The listing builds one solid part. Answer for the finished solid, in the listing's coordinates (mm). A direction names the side the tool comes from. Give positions to 0.01 mm unless a question says otherwise; leave off trailing zeros. Loops run counter-clockwise (first coordinate to the right, second up) from the corner with the lowest first, then second, coordinate; pieces in that order, holes last. Notation, with made-up numbers: M -18.5,31.25 L 32.5,31.25 A20 ccw 32.5,45.25 Z; hole C -6.75,76.25 d4. An arc over 180 degrees is marked long. One line per item, written item: value. Start each with the question number.
Q1. A cutting plane is placed at D-D, the plane z = -24. Determine the outline of the cut face in (x, y).
Q2. A cutting plane is placed at C-C, the plane x = 82. Determine the outline of the cut face in (y, z).
Q3. A cutting plane is placed at B-B, the plane y = 4. State how many separate pieces and enclosed holes the cut face has, and give its area (3 significant figures).
Q4. Consider L1, parallel to X at y = -20, z = 0; L2, parallel to Z at x = -11, y = 2.5; L3, parallel to X at y = -26, z = 4. Determine where each line is inside the solid, lowest interval first.
Q5. The mould has two halves that part along X. Classify faces 4 (the flat face through (90, -12, 0)), 5 (the flat face through (24, -4, -20)), 6 (the cylindrical face through (67.436, -17.675, 0.976)): +X half, -X half, draft (parallel to the pull), parting line (faces both ways), or undercut.
Q6. For faces 1 (the flat face through (26, -20, -24)), 2 (the flat face through (32, 2, 0)), 3 (the cylindrical face through (-17.32, -17.68, 1.63)), determine the directions among +Z, -Z, +X, -X, +Y, -Y from which every point of the face is accessible in a straight line to the end or side of a thin tool.
Q7. A cutting plane is placed at A-A, the plane y = -22. Determine the outline of the cut face in (x, z), and give its area (3 significant figures).
Q8. Flat-ended cylindrical pins translate along their axes: pin 1 (19.5 mm diameter, centred on x = 60, z = 0, fed in from +Y); pin 2 (1 mm diameter, centred on x = 24, y = -23, fed in from -Z); pin 3 (2 mm diameter, centred on x = 39, z = -23.5, fed in from +Y); pin 4 (3 mm diameter, centred on x = 54, y = -22.5, fed in from +Z). Find the tip coordinate at first contact, or state that the pin passes through.
from build123d import *

# Parameters (mm, degrees)
SKETCH1_W           = 180
SKETCH1_H           = 40
BOSS_EXTRUDE1_DEPTH = 6
CUT_EXTRUDE2_DEPTH  = 4
SKETCH6_W           = 180
SKETCH6_H           = 40
BOSS_EXTRUDE3_DEPTH = 30
SKETCH7_W           = 50
SKETCH7_H           = 40
CUT_EXTRUDE3_DEPTH  = 40
SKETCH8_W           = 55
SKETCH8_H           = 10
BOSS_EXTRUDE4_DEPTH = 130
SKETCH9_R           = 7.5
CUT_EXTRUDE4_DEPTH  = 25


with BuildPart() as part:
    # Sketch1 → Boss-Extrude1 (new body)
    with BuildSketch(Plane(origin=(0, 0, 0), x_dir=(1, 0, 0), z_dir=(0, 1, 0))):
        Rectangle(SKETCH1_W, SKETCH1_H)
    extrude(amount=BOSS_EXTRUDE1_DEPTH)

    # Sketch5 → Cut-Extrude2 (cut)
    with BuildSketch(Plane(origin=(0, 6, 0), x_dir=(1, 0, 0), z_dir=(0, 1, 0))):
        with BuildLine():
            Line((-105.561478508, 98.797927369), (119.027484656, -125.791035795))
            ThreePointArc((119.027484656, -125.791035795), (119.027484656, -129.326569701), (115.49195075, -129.326569701))
            Line((115.49195075, -129.326569701), (-109.097012414, 95.262393463))
            ThreePointArc((-109.097012414, 95.262393463), (-109.097012414, 98.797927369), (-105.561478508, 98.797927369))
        make_face()
        with BuildLine():
            Line((-102.025944602, 102.333461275), (122.563018562, -122.255501889))
            ThreePointArc((122.563018562, -122.255501889), (126.098552468, -122.255501889), (126.098552468, -118.719967983))
            Line((126.098552468, -118.719967983), (-98.490410696, 105.868995181))
            ThreePointArc((-98.490410696, 105.868995181), (-102.025944602, 105.868995181), (-102.025944602, 102.333461275))
        make_face()
        with BuildLine():
            Line((-94.95487679, 109.404529087), (129.634086374, -115.184434077))
            ThreePointArc((129.634086374, -115.184434077), (133.16962028, -115.184434077), (133.16962028, -111.648900171))
            Line((133.16962028, -111.648900171), (-91.419342885, 112.940062993))
            ThreePointArc((-91.419342885, 112.940062993), (-94.95487679, 112.940062993), (-94.95487679, 109.404529087))
        make_face()
        with BuildLine():
            Line((-87.883808979, 116.475596899), (136.705154185, -108.113366265))
            ThreePointArc((136.705154185, -108.113366265), (140.240688091, -108.113366265), (140.240688091, -104.577832359))
            Line((140.240688091, -104.577832359), (-84.348275073, 120.011130805))
            ThreePointArc((-84.348275073, 120.011130805), (-87.883808979, 120.011130805), (-87.883808979, 116.475596899))
        make_face()
        with BuildLine():
            Line((-80.812741167, 123.546664711), (143.776221997, -101.042298453))
            ThreePointArc((143.776221997, -101.042298453), (147.311755903, -101.042298453), (147.311755903, -97.506764547))
            Line((147.311755903, -97.506764547), (-77.277207261, 127.082198617))
            ThreePointArc((-77.277207261, 127.082198617), (-80.812741167, 127.082198617), (-80.812741167, 123.546664711))
        make_face()
        with BuildLine():
            Line((-73.741673355, 130.617732523), (150.847289809, -93.971230641))
            ThreePointArc((150.847289809, -93.971230641), (154.382823715, -93.971230641), (154.382823715, -90.435696735))
            Line((154.382823715, -90.435696735), (-70.206139449, 134.153266429))
            ThreePointArc((-70.206139449, 134.153266429), (-73.741673355, 134.153266429), (-73.741673355, 130.617732523))
        make_face()
        with BuildLine():
            Line((-66.670605543, 137.688800335), (157.918357621, -86.900162829))
            ThreePointArc((157.918357621, -86.900162829), (161.453891527, -86.900162829), (161.453891527, -83.364628923))
            Line((161.453891527, -83.364628923), (-63.135071637, 141.224334241))
            ThreePointArc((-63.135071637, 141.224334241), (-66.670605543, 141.224334241), (-66.670605543, 137.688800335))
        make_face()
        with BuildLine():
            Line((-59.599537731, 144.759868147), (164.989425433, -79.829095018))
            ThreePointArc((164.989425433, -79.829095018), (168.524959339, -79.829095018), (168.524959339, -76.293561112))
            Line((168.524959339, -76.293561112), (-56.064003825, 148.295402052))
            ThreePointArc((-56.064003825, 148.295402052), (-59.599537731, 148.295402052), (-59.599537731, 144.759868147))
        make_face()
        with BuildLine():
            Line((-52.528469919, 151.830935958), (172.060493245, -72.758027206))
            ThreePointArc((172.060493245, -72.758027206), (175.596027151, -72.758027206), (175.596027151, -69.2224933))
            Line((175.596027151, -69.2224933), (-48.992936013, 155.366469864))
            ThreePointArc((-48.992936013, 155.366469864), (-52.528469919, 155.366469864), (-52.528469919, 151.830935958))
        make_face()
        with BuildLine():
            Line((-45.457402107, 158.90200377), (179.131561057, -65.686959394))
            ThreePointArc((179.131561057, -65.686959394), (182.667094963, -65.686959394), (182.667094963, -62.151425488))
            Line((182.667094963, -62.151425488), (-41.921868201, 162.437537676))
            ThreePointArc((-41.921868201, 162.437537676), (-45.457402107, 162.437537676), (-45.457402107, 158.90200377))
        make_face()
        with BuildLine():
            Line((-116.168080226, 88.191325652), (108.420882938, -136.397637512))
            ThreePointArc((108.420882938, -136.397637512), (111.956416844, -136.397637512), (111.956416844, -132.862103607))
            Line((111.956416844, -132.862103607), (-112.63254632, 91.726859558))
            ThreePointArc((-112.63254632, 91.726859558), (-116.168080226, 91.726859558), (-116.168080226, 88.191325652))
        make_face()
        with BuildLine():
            Line((-123.239148038, 81.12025784), (101.349815126, -143.468705324))
            ThreePointArc((101.349815126, -143.468705324), (104.885349032, -143.468705324), (104.885349032, -139.933171418))
            Line((104.885349032, -139.933171418), (-119.703614132, 84.655791746))
            ThreePointArc((-119.703614132, 84.655791746), (-123.239148038, 84.655791746), (-123.239148038, 81.12025784))
        make_face()
        with BuildLine():
            Line((-130.31021585, 74.049190028), (94.278747314, -150.539773136))
            ThreePointArc((94.278747314, -150.539773136), (97.81428122, -150.539773136), (97.81428122, -147.00423923))
            Line((97.81428122, -147.00423923), (-126.774681944, 77.584723934))
            ThreePointArc((-126.774681944, 77.584723934), (-130.31021585, 77.584723934), (-130.31021585, 74.049190028))
        make_face()
        with BuildLine():
            Line((-137.381283662, 66.978122216), (87.207679502, -157.610840948))
            ThreePointArc((87.207679502, -157.610840948), (90.743213408, -157.610840948), (90.743213408, -154.075307042))
            Line((90.743213408, -154.075307042), (-133.845749756, 70.513656122))
            ThreePointArc((-133.845749756, 70.513656122), (-137.381283662, 70.513656122), (-137.381283662, 66.978122216))
        make_face()
        with BuildLine():
            Line((-144.452351474, 59.907054404), (80.136611691, -164.68190876))
            ThreePointArc((80.136611691, -164.68190876), (83.672145596, -164.68190876), (83.672145596, -161.146374854))
            Line((83.672145596, -161.146374854), (-140.916817568, 63.44258831))
            ThreePointArc((-140.916817568, 63.44258831), (-144.452351474, 63.44258831), (-144.452351474, 59.907054404))
        make_face()
        with BuildLine():
            Line((-151.523419285, 52.835986592), (73.065543879, -171.752976572))
            ThreePointArc((73.065543879, -171.752976572), (76.601077785, -171.752976572), (76.601077785, -168.217442666))
            Line((76.601077785, -168.217442666), (-147.987885379, 56.371520498))
            ThreePointArc((-147.987885379, 56.371520498), (-151.523419285, 56.371520498), (-151.523419285, 52.835986592))
        make_face()
        with BuildLine():
            Line((-158.594487097, 45.76491878), (65.994476067, -178.824044384))
            ThreePointArc((65.994476067, -178.824044384), (69.530009973, -178.824044384), (69.530009973, -175.288510478))
            Line((69.530009973, -175.288510478), (-155.058953191, 49.300452686))
            ThreePointArc((-155.058953191, 49.300452686), (-158.594487097, 49.300452686), (-158.594487097, 45.76491878))
        make_face()
    extrude(amount=-CUT_EXTRUDE2_DEPTH, mode=Mode.SUBTRACT)

    # Sketch6 → Boss-Extrude3 (add)
    with BuildSketch(Plane.XZ):
        Rectangle(SKETCH6_W, SKETCH6_H)
    extrude(amount=BOSS_EXTRUDE3_DEPTH)

    # Sketch7 → Cut-Extrude3 (cut)
    with BuildSketch(Plane.XZ.offset(30)):
        with Locations((-65, 0)):
            Rectangle(SKETCH7_W, SKETCH7_H)
    extrude(amount=-CUT_EXTRUDE3_DEPTH, mode=Mode.SUBTRACT)

    # Sketch8 → Boss-Extrude4 (add, through all)
    with BuildSketch(Plane(origin=(90, 0, 0), x_dir=(0, 0, -1), z_dir=(1, 0, 0))):
        with Locations((0, -15)):
            Rectangle(SKETCH8_W, SKETCH8_H)
    extrude(amount=-BOSS_EXTRUDE4_DEPTH)

    # Sketch9 → Cut-Extrude4 (cut)
    with BuildSketch(Plane.XZ.offset(30)):
        with Locations(Location((60, 0, 0), (0, 0, 270))):
            Circle(SKETCH9_R)
        with Locations(Location((-10, 0, 0), (0, 0, 270))):
            Circle(SKETCH9_R)
    extrude(amount=-CUT_EXTRUDE4_DEPTH, mode=Mode.SUBTRACT)


solid = part.part
Answer block:
1. outline: M -40,-20 L 90,-20 L 90,-10 L -40,-10 Z
2. outline: M -30,-20 L -20,-20 L -20,-27.5 L -10,-27.5 L -10,-20 L 2,-20 L 2,-17.3 L 6,-17.3 L 6,-10.23 L 2,-10.23 L 2,-3.16 L 6,-3.16 L 6,3.91 L 2,3.91 L 2,10.98 L 6,10.98 L 6,18.05 L 2,18.05 L 2,20 L -10,20 L -10,27.5 L -20,27.5 L -20,20 L -30,20 Z
3. separate pieces: 13
3. enclosed holes: 0
3. area: 2,600 mm^2
4. L1: -40 to -17.5, -2.5 to 52.5, 67.5 to 90
4. L2: -20 to -18.38, -11.31 to -4.24, 2.83 to 9.91, 16.98 to 20
4. L3: -40 to -16.34, -3.66 to 53.66, 66.34 to 90
5. face 4: +X half
5. face 5: draft
5. face 6: undercut
6. face 1: -Z, +X, -X, -Y
6. face 2: +Y
6. face 3: -Y
7. outline: M -40,-20 L 90,-20 L 90,20 L -40,20 Z; hole C -10,0 d15; hole C 60,0 d15
7. area: 4,850 mm^2
8. pin 1: y = 6
8. pin 2: z = -20
8. pin 3: y = -10
8. pin 4: z = 20
